Part print with two shaded views. Sizes in mm from the minimum x, y, z corner. Give positions to 0.01 mm unless a question says otherwise; leave off trailing zeros. Order: outer loops, then holes, each group sorted by start corner. A loop starts at its lowest first (then second) coordinate and runs counter-clockwise, first axis right, second up. Notation, with made-up numbers: M 33,77.5 L 42,77.5 A16 ccw 42,105.5 Z; hole C 82,4.25 d5. An arc over 180 degrees is marked long. Return JSON: item names as keys, results as strings. Group by question number.
1. Slice it at B-B on y = 103.5. List the corners of the cut face in (x, z).
2. Slice it at A-A on z = 1.15. Give the number of separate pieces and of enclosed holes in the cut face, then the cut area to 3 significant figures.
3. Wall check: probe 1 along X at (y, z) = (215, 1.95); probe 2 along Y at (x, z) = (25, 2.95); probe 3 along Y at (x, z) = (10, 1.8). Give the ranges that are in metal, low to high. Write a range as [from, to].
4. Pin check, flat tips, straight feed: pin 1 (2.5 mm diameter, centred on x = 33.5, z = 3.5, fed in from +Y); pin 2 (2.5 mm diameter, centred on y = 121, z = 2, fed in from +X). Stop position of each tip, or through.
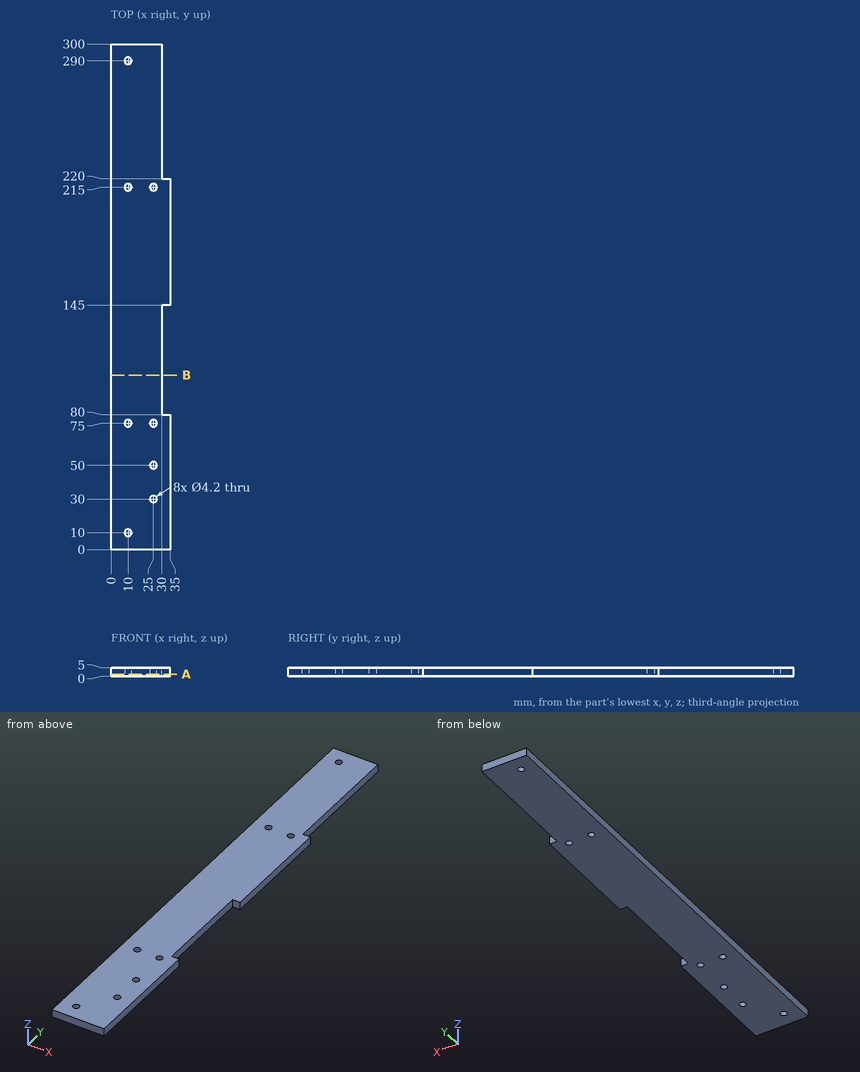
Result:
{
 "1": {"outline": "M 0,0 L 30,0 L 30,5 L 0,5 Z"},
 "2": {"separate pieces": "1", "enclosed holes": "8", "area": "9,660 mm2"},
 "3": {"probe 1": "x = [0, 7.9], [12.1, 22.9], [27.1, 35]", "probe 2": "y = [0, 27.9], [32.1, 47.9], [52.1, 72.9], [77.1, 212.9], [217.1, 300]", "probe 3": "y = [0, 7.9], [12.1, 72.9], [77.1, 212.9], [217.1, 287.9], [292.1, 300]"},
 "4": {"pin 1": "stops at y = 220", "pin 2": "stops at x = 30"}
}
